Design review of the part built by this model. Coordinates are the model's own, in mm. Round coordinates to 2 decimals unless told otherwise and drop trailing zeros. Order: outer loops, then holes, each group sorted by start corner. A loop starts at its lowest first (then second) coordinate and runs counter-clockwise, first axis right, second up. Notation, with made-up numbers: M -29.75,43.5 L -7.75,43.5 A23 ccw -7.75,71.5 Z; hole C 55.25,64.25 d2. An arc over 180 degrees is marked long. Use a Markdown table: item, result. Add a question column.
(1) Take a section at B-B (z = -5.25). Write out the cut boundary in (x, y).
(2) Take a section at A-A (x = 123.5). Write out the cut boundary in (y, z), then the cut area to 3 significant figures.
(3) To check wall thickness, follow probe 1 along Y at (x, z) = (225.5, -8.25); probe 2 along Y at (x, z) = (241, -7.25); probe 3 along Y at (x, z) = (162.5, -4.5). State the ranges of each line that lie inside material, in increasing order. Write a range as from..to.
(4) Take a section at C-C (y = 66.5). Write out the cut boundary in (x, z).
(5) For pin 1 (2 mm diameter, centred on y = 54.5, z = -8, fed in from -X); pin 2 (10.5 mm diameter, centred on x = 162.9, y = 320.19, fed in from -Z); pin 3 (5 mm diameter, centred on x = 203.41, y = 349.1, fed in from -Z); pin 4 (5 mm diameter, centred on x = 270, z = -3, fed in from +Y), all flat-tipped, find the tip position at first contact; note any pin that passes through.
(6) Take a section at D-D (x = 178.5). Write out the cut boundary in (y, z), then the cut area to 3 significant figures.
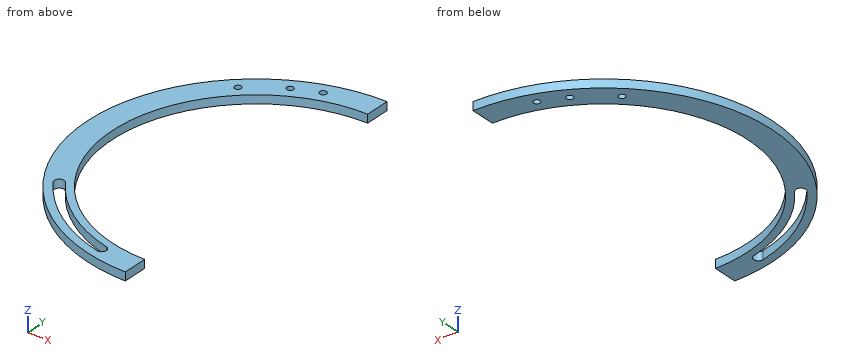
```python
from build123d import *

# Parameters (mm, degrees)
SKETCH1_R               = 203.294925519
SKETCH1_R_2             = 173.294925519
BOSS_EXTRUDE1_DEPTH     = 10
CUT_EXTRUDE1_START      = -185
CUT_EXTRUDE1_DEPTH      = 185
CUT_EXTRUDE2_DEPTH      = 185
CUT_EXTRUDE3_DEPTH      = 484.877792972
CUT_EXTRUDE3_DEPTH_BACK = 484.877792972
SKETCH4_R               = 4


with BuildPart() as part:
    # Sketch1 → Boss-Extrude1 (new body)
    with BuildSketch(Plane.XY):
        with Locations((291.585214163, 182.730697222)):
            Circle(SKETCH1_R)
        with Locations((291.585214163, 182.730697222)):
            Circle(SKETCH1_R_2, mode=Mode.SUBTRACT)
    extrude(amount=-BOSS_EXTRUDE1_DEPTH)

    # Sketch2 → Cut-Extrude1 (cut)
    with BuildSketch(Plane(origin=(0, 0, -10), x_dir=(-1, 0, 0), z_dir=(0, 0, -1)).offset(CUT_EXTRUDE1_START)):
        with BuildLine():
            Line((-291.585214163, 9.435771703), (-291.585214163, -33.905509081))
            ThreePointArc((-291.585214163, -33.905509081), (-508.221420466, 182.730697222), (-291.585214163, 399.366903525))
            Line((-291.585214163, 399.366903525), (-291.585214163, 356.025622742))
            ThreePointArc((-291.585214163, 356.025622742), (-464.880139683, 182.730697222), (-291.585214163, 9.435771703))
        make_face()
    extrude(amount=CUT_EXTRUDE1_DEPTH, mode=Mode.SUBTRACT)

    # Sketch3 → Cut-Extrude2 (cut)
    with BuildSketch(Plane(origin=(0, 0, -10), x_dir=(-1, 0, 0), z_dir=(0, 0, -1))):
        with BuildLine():
            ThreePointArc((-245.463287057, -5.419646314), (-182.427275621, 22.692175653), (-133.247878722, 71.11944269))
            ThreePointArc((-133.247878722, 71.11944269), (-134.651744503, 79.229936459), (-142.762238272, 77.826070678))
            ThreePointArc((-142.762238272, 77.826070678), (-188.98648588, 32.30875807), (-248.234715516, 5.886152238))
            ThreePointArc((-248.234715516, 5.886152238), (-252.501900562, -1.152461267), (-245.463287057, -5.419646314))
        make_face()
    extrude(amount=-CUT_EXTRUDE2_DEPTH, mode=Mode.SUBTRACT)

    # Sketch4 → Cut-Extrude3 (cut, two sides: drawn at the far end of the back side and taken through both)
    with BuildSketch(Plane(origin=(0, 0, -10), x_dir=(-1, 0, 0), z_dir=(0, 0, -1)).offset(-CUT_EXTRUDE3_DEPTH_BACK)):
        with Locations((-203.411601384, 349.104953001)):
            Circle(SKETCH4_R)
        with Locations((-233.317748738, 361.783430933)):
            Circle(SKETCH4_R)
        with Locations((-162.898022452, 320.188274917)):
            Circle(SKETCH4_R)
    extrude(amount=CUT_EXTRUDE3_DEPTH + CUT_EXTRUDE3_DEPTH_BACK, mode=Mode.SUBTRACT)


solid = part.part
```
Verdict:
| question | item | result |
|---|---|---|
| 1 | outline | M 291.59,-20.56 L 291.59,9.44 A173.29 cw 291.59,356.03 L 291.59,386.03 A203.29 ccw Z; hole M 133.25,71.12 A193.72 ccw 245.46,-5.42 A5.82 ccw 248.23,5.89 A182.08 cw 142.76,77.83 A5.82 ccw Z; hole C 162.9,320.19 d8; hole C 203.41,349.1 d8; hole C 233.32,361.78 d8 |
| 2 | outline | M 68.38,-10 L 140.56,-10 L 140.56,0 L 68.38,0 Z; M 224.9,-10 L 297.08,-10 L 297.08,0 L 224.9,0 Z |
| 2 | area | 1,440 mm^2 |
| 3 | probe 1 | y = -9.52..0.63, 13.07..22.53, 342.93..374.98 |
| 3 | probe 2 | y = -14.17..-4.27, 7.82..16.98, 348.48..379.63 |
| 3 | probe 3 | y = 25.68..38.28, 54.32..67.11, 298.35..316.21, 324.17..339.78 |
| 4 | outline | M 124.79,-10 L 136.61,-10 L 136.61,0 L 124.79,0 Z; M 151.43,-10 L 163.05,-10 L 163.05,0 L 151.43,0 Z |
| 5 | pin 1 | stops at x = 133.03 |
| 5 | pin 2 | stops at z = -10 |
| 5 | pin 3 | passes through |
| 5 | pin 4 | stops at y = 385.13 |
| 6 | outline | M 13.79,-10 L 25.44,-10 L 25.44,0 L 13.79,0 Z; M 40.02,-10 L 51.42,-10 L 51.42,0 L 40.02,0 Z; M 314.04,-10 L 351.67,-10 L 351.67,0 L 314.04,0 Z |
| 6 | area | 607 mm^2 |
